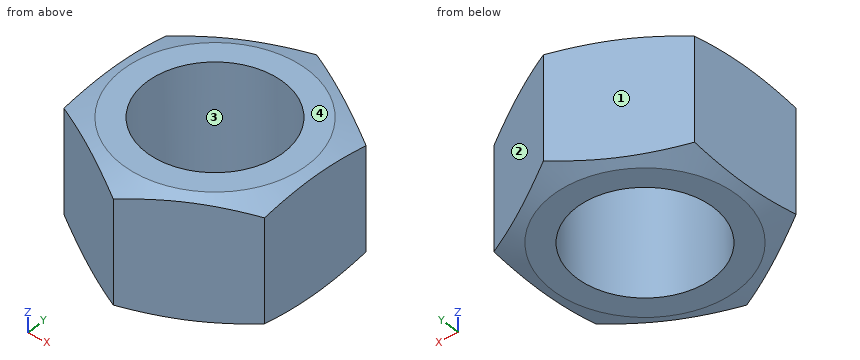
from build123d import *

# Parameters (mm, degrees)
BOSS_EXTRUDE1_DEPTH = 10.8
SKETCH5_R           = 6
CUT_EXTRUDE1_DEPTH  = 18.482562742


with BuildPart() as part:
    # Sketch1 → Boss-Extrude1 (new body)
    with BuildSketch(Plane.XY):
        Polygon((0, 10.392304845), (-9, 5.196152423), (-9, -5.196152423), (0, -10.392304845), (9, -5.196152423), (9, 5.196152423), align=None)
    extrude(amount=BOSS_EXTRUDE1_DEPTH)

    # Sketch4 → Cut-Revolve1 (revolve, cut)
    with BuildSketch(Plane(origin=(0, 0, 0), x_dir=(0, 0, -1), z_dir=(1, 0, 0)), mode=Mode.PRIVATE) as cut_revolve1_sk:
        Polygon((-10.8, -8.1), (-9.965669268, -10.392304845), (-10.8, -10.392304845), align=None)
    cut_revolve1 = revolve(cut_revolve1_sk.sketch.rotate(Axis((0, 0, 10.8), (0, 0, -1)), 119.999999988), axis=Axis((0, 0, 10.8), (0, 0, -1)), mode=Mode.SUBTRACT)

    # Mirror1: Cut-Revolve1 across plane
    add(cut_revolve1.mirror(Plane.XY.offset(5.4)), mode=Mode.SUBTRACT)

    # Sketch5 → Cut-Extrude1 (cut, through all)
    with BuildSketch(Plane.XY.offset(10.8)):
        Circle(SKETCH5_R)
    extrude(amount=-CUT_EXTRUDE1_DEPTH, mode=Mode.SUBTRACT)


solid = part.part
Read the model definition and answer for the solid it produces. Units are mm, in the model's axes. Face numbers are marked on the shaded views. Coordinates: 2 decimals unless noted, no trailing zeros. Write each loop counter-clockwise with the first axis right and the second up, starting at its lowest first coordinate (ties: lowest second). Pieces come first, ordered by that corner, then holes. Notation, with made-up numbers: (49, 83.5) -> (73, 83.5) arc R24 cw to (73, 109.5) -> close; hole circle Ø3 at (71, -9). An arc over 180 degrees is marked (long way). Return JSON: item names as keys, results as strings.
(1) Each of these flat-tipped pins is pushed along its axis until it touches: P1, Ø5, axis at x = 0.5, z = 4, coming from the +Y side; P2, Ø2, axis at y = -8, z = 5.5, coming from the -X side; P3, Ø1.5, axis at x = 3.5, z = 2.5, coming from the +Y side. Where does it stop, or does it pass through?
Answers below:
{"P1": "y = 10.39", "P2": "x = -5.88", "P3": "y = 8.8"}
(2) The part is cut by section A-A on y = 0. Give the vertices of the cut face in (x, z).
Answers below:
{"outline": "(-9, 0.33) -> (-8.1, 0) -> (-6, 0) -> (-6, 10.8) -> (-8.1, 10.8) -> (-9, 10.47) -> close; (6, 0) -> (8.1, 0) -> (9, 0.33) -> (9, 10.47) -> (8.1, 10.8) -> (6, 10.8) -> close"}
(3) The part is cut by section B-B on z = 3.75. Give the vertices of the cut face in (x, y), then the cut area to 3 significant figures.
Answers below:
{"outline": "(-9, -5.2) -> (0, -10.39) -> (9, -5.2) -> (9, 5.2) -> (0, 10.39) -> (-9, 5.2) -> close; hole circle Ø12 at (0, 0)", "area": "167 mm^2"}
(4) For a pull along X with two mould halves and no side action, classify the marked faces 1, 2, 3 and 4 as pulls with the +X half, pulls with the -X half, needs draft (parallel to the pull), parting line crosses it, or undercut.
Answers below:
{"face 1": "pulls with the -X half", "face 2": "pulls with the +X half", "face 3": "undercut", "face 4": "needs draft"}
(5) Consider line 1 along X through (y, z) = (-3, 7.5); line 2 along Y through (x, z) = (1.5, 8); line 3 along Y through (x, z) = (3.75, 4.25). Determine where each line is inside the solid, lowest interval first. Write a range as from..to.
Answers below:
{"line 1": "-9..-5.2, 5.2..9", "line 2": "-9.53..-5.81, 5.81..9.53", "line 3": "-8.23..-4.68, 4.68..8.23"}
